Part model, mm, in its own coordinate system. Face numbers are marked on the shaded views. A direction names the side the tool comes from. Coordinates: 2 decimals unless noted, no trailing zeros. Write each loop counter-clockwise with the first axis right and the second up, starting at its lowest first coordinate (ties: lowest second). Pieces come first, ordered by that corner, then holes. Notation, with made-up numbers: (68, -4) -> (91, -4) arc R23 ccw to (91, 32) -> close; hole circle Ø1 at (13, 15.5). An arc over 180 degrees is marked (long way). Write item = value, one per line. Start each with the question number.
Q1. Tool access for the marked faces 4 and 5: list every direction of +Z, -Z, +X, -X, +Y, -Y with a clear straight run to the whole face (end or side of a thin tool).
Q2. Band-saw the part on A-A, the plane z = 59. List the corners of the cut face in (x, y), plus the area to 3 significant figures.
Q3. Band-saw the part on B-B, the plane y = -45. List the corners of the cut face in (x, z).
Q4. Probe line 1 (Z direction, x = 20.5, y = -40.5); line 2 (Y direction, x = 31.5, z = 42). List the from-to ranges inside material, lowest first.
Q5. Pull direction Z, two halves, no side cores. Call the marked faces 1, 2 and 3: released by +Z, released by -Z, zero draft, split by the parting line, or undercut.
Q6. Band-saw the part on C-C, the plane x = -12. List the corners of the cut face in (y, z).
Q7. Band-saw the part on D-D, the plane z = -45. List the corners of the cut face in (x, y).
Q8. Pin check, flat tips, straight feed: P1, Ø1.5, axis at x = -7.5, y = -78, coming from the -Z side; P2, Ø0.9, axis at x = 122.5, y = -79, coming from the -Z side; P3, Ø2.5, axis at x = 122, y = -79, coming from the +Z side. Stop position of each tip, or through.
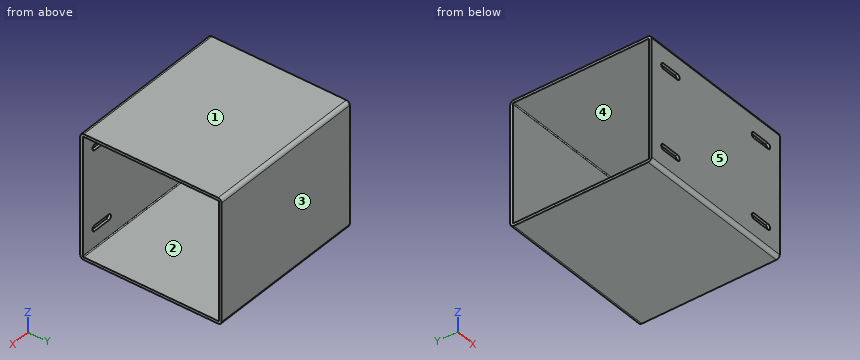
from build123d import *

# Parameters (mm, degrees)
EXTRUDE_1_DEPTH      = 150
EXTRUDE_1_DEPTH_BACK = 34
SKETCH_2_W           = 140
SKETCH_2_H           = 160
SKETCH_2_W_2         = 134
SKETCH_2_H_2         = 154
CUT_EXTRUDE_1_DEPTH  = 10
FILLET_1_R           = 1
FILLET_2_R           = 4


with BuildPart() as part:
    # 草图2 → 凸台-拉伸1 (new, two sides: drawn at the far end of the back side and taken through both)
    with BuildSketch(Plane(origin=(0, 0, 0), x_dir=(0, 0, -1), z_dir=(1, 0, 0)).offset(-EXTRUDE_1_DEPTH_BACK)):
        Rectangle(SKETCH_2_W, SKETCH_2_H)
        Rectangle(SKETCH_2_W_2, SKETCH_2_H_2, mode=Mode.SUBTRACT)
    extrude(amount=EXTRUDE_1_DEPTH + EXTRUDE_1_DEPTH_BACK)

    # 草图3 → 切除-拉伸1 (cut)
    with BuildSketch(Plane(origin=(0, -77, 0), x_dir=(1, 0, 0), z_dir=(0, 1, 0))):
        with BuildLine():
            Line((-17, 48.25), (3, 48.25))
            ThreePointArc((3, 48.25), (6.25, 45), (3, 41.75))
            Line((3, 41.75), (-17, 41.75))
            ThreePointArc((-17, 41.75), (-20.25, 45), (-17, 48.25))
        make_face()
        with BuildLine():
            Line((-17, -48.25), (3, -48.25))
            ThreePointArc((3, -48.25), (6.25, -45), (3, -41.75))
            Line((3, -41.75), (-17, -41.75))
            ThreePointArc((-17, -41.75), (-20.25, -45), (-17, -48.25))
        make_face()
        with BuildLine():
            Line((133, 48.25), (113, 48.25))
            ThreePointArc((113, 48.25), (109.75, 45), (113, 41.75))
            Line((113, 41.75), (133, 41.75))
            ThreePointArc((133, 41.75), (136.25, 45), (133, 48.25))
        make_face()
        with BuildLine():
            Line((133, -48.25), (113, -48.25))
            ThreePointArc((113, -48.25), (109.75, -45), (113, -41.75))
            Line((113, -41.75), (133, -41.75))
            ThreePointArc((133, -41.75), (136.25, -45), (133, -48.25))
        make_face()
    extrude(amount=-CUT_EXTRUDE_1_DEPTH, mode=Mode.SUBTRACT)

    # 圆角1
    fillet_1_edges = [part.edges().sort_by_distance(p)[0] for p in [
        (58, -77, 67),
        (58, 77, 67),
        (58, 77, -67),
        (58, -77, -67),
    ]]
    fillet(fillet_1_edges, radius=FILLET_1_R)

    # 圆角2
    fillet_2_edges = [part.edges().sort_by_distance(p)[0] for p in [
        (58, -80, -70),
        (58, -80, 70),
        (58, 80, 70),
        (58, 80, -70),
    ]]
    fillet(fillet_2_edges, radius=FILLET_2_R)


solid = part.part
Ans:
q1.face_4 = +X, -X
q1.face_5 = +Z, -Z, +X, -X, -Y
q2.outline = (-34, -80) -> (150, -80) -> (150, -77) -> (-34, -77) -> close; (-34, 77) -> (150, 77) -> (150, 80) -> (-34, 80) -> close
q2.area = 1,100 mm2
q3.outline = (-34, -70) -> (150, -70) -> (150, -67) -> (-34, -67) -> close; (-34, 67) -> (150, 67) -> (150, 70) -> (-34, 70) -> close
q4.line_1 = -70 to -67, 67 to 70
q4.line_2 = -80 to -77, 77 to 80
q5.face_1 = released by +Z
q5.face_2 = undercut
q5.face_3 = zero draft
q6.outline = (-80, -66) arc R4 ccw to (-76, -70) -> (76, -70) arc R4 ccw to (80, -66) -> (80, 66) arc R4 ccw to (76, 70) -> (-76, 70) arc R4 ccw to (-80, 66) -> (-80, 48.25) -> (-77, 48.25) -> (-77, 66) arc R1 cw to (-76, 67) -> (76, 67) arc R1 cw to (77, 66) -> (77, -66) arc R1 cw to (76, -67) -> (-76, -67) arc R1 cw to (-77, -66) -> (-77, -48.25) -> (-80, -48.25) -> close; (-80, -41.75) -> (-77, -41.75) -> (-77, 41.75) -> (-80, 41.75) -> close
q7.outline = (-34, -80) -> (-20.25, -80) -> (-20.25, -77) -> (-34, -77) -> close; (-34, 77) -> (150, 77) -> (150, 80) -> (-34, 80) -> close; (6.25, -80) -> (109.75, -80) -> (109.75, -77) -> (6.25, -77) -> close; (136.25, -80) -> (150, -80) -> (150, -77) -> (136.25, -77) -> close
q8.P1 = -69.8
q8.P2 = -69.08
q8.P3 = 69.6
